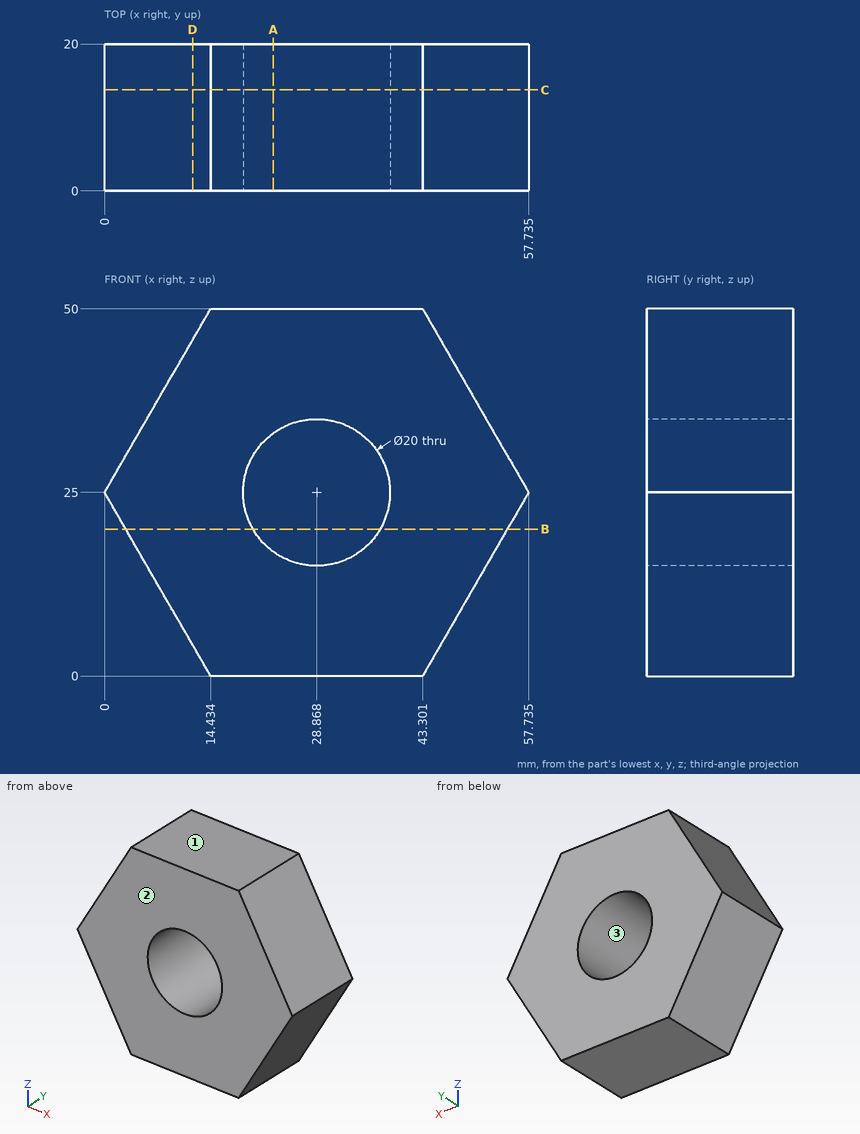
Design review of the part shown in the three views and the two pictorial views. Dimensions are in mm from the part's minimum x, y and z. Round coordinates to 2 decimals unless told otherwise and drop trailing zeros. Write each loop counter-clockwise with the first axis right and the second up, starting at its lowest first coordinate (ties: lowest second). Pieces come first, ordered by that corner, then holes.
Item 1: We need section B-B on z = 20. Write out the cut boundary in (x, y), and give its area (3 significant figures).
Item 2: The part is to be moulded in two halves that separate along Z. For the marked faces 1, 2 and 3, say which applies: +Z half, -Z half, draft (parallel to the pull), parting line (faces both ways), or undercut.
Item 3: We need section C-C on y = 13.75. Write out the cut boundary in (x, z) (1 decimal).
Item 4: We need section A-A on x = 23. Write out the cut boundary in (y, z), and give its area (3 significant figures).
Item 5: For probe 1 along Z at (x, y) = (34, 2.5); probe 2 along X at (y, z) = (10, 17) (1 decimal); probe 3 along X at (y, z) = (11, 23) (1 decimal), list the stretches that pass through material, from the lowest coordinate up.
Item 6: We need section D-D on x = 12. Write out the cut boundary in (y, z) (1 decimal).
Item 7: Clearance check with flat-ended pins moving along their axes: pin 1 Ø6 at (x, y) = (9.5, 4.5) entering from +Z; pin 2 Ø8 at (x, y) = (48.5, 4) entering from -Z (1 decimal); pin 3 Ø6 at (y, z) = (5, 40.5) entering from -X; pin 4 Ø16 at (x, z) = (28.87, 25) entering from -Y. State where each tip first meets the part, or that it passes through.
Returned:
1. outline: (2.89, 0) - (20.21, 0) - (20.21, 20) - (2.89, 20) - close; (37.53, 0) - (54.85, 0) - (54.85, 20) - (37.53, 20) - close
1. area: 693 mm2
2. face 1: +Z half
2. face 2: draft
2. face 3: undercut
3. outline: (0, 25) - (14.4, 0) - (43.3, 0) - (57.7, 25) - (43.3, 50) - (14.4, 50) - close; hole circle Ø20 at (28.9, 25)
4. outline: (0, 0) - (20, 0) - (20, 16.9) - (0, 16.9) - close; (0, 33.1) - (20, 33.1) - (20, 50) - (0, 50) - close
4. area: 676 mm2
5. probe 1: z = 0 to 16.42, 33.58 to 50
5. probe 2: x = 4.6 to 22.9, 34.9 to 53.1
5. probe 3: x = 1.2 to 19.1, 38.7 to 56.6
6. outline: (0, 4.2) - (20, 4.2) - (20, 45.8) - (0, 45.8) - close
7. pin 1: stops at z = 46.65
7. pin 2: stops at z = 2.1
7. pin 3: stops at x = 7.22
7. pin 4: passes through
